The model under review builds one solid part; all positions refer to its coordinate system, in mm. Give positions to 0.01 mm unless a question says otherwise; leave off trailing zeros. Order: outer loops, then holes, each group sorted by start corner. A loop starts at its lowest first (then second) coordinate and runs counter-clockwise, first axis right, second up. Notation, with made-up numbers: (-18, 0.25) - (23, 0.25) arc R17 ccw to (23, 32.25) - close; hole circle Ø7 at (13.25, 10). An arc over 180 degrees is marked (long way). Use CSV: the item, a comma, the result in double quotes.
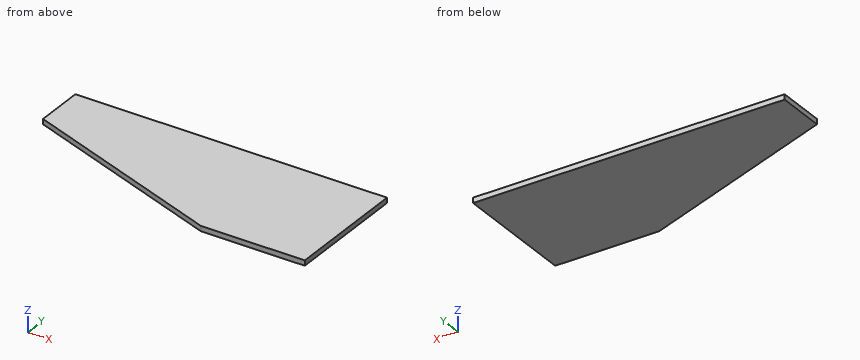
```python
from build123d import *

# Parameters (mm, degrees)
EXTRUDE_1_DEPTH = 5


with BuildPart() as part:
    # 草图1 → 凸台-拉伸1 (new body)
    with BuildSketch(Plane.XY):
        Polygon((0, 0), (300, 0), (300, -120), (200, -120), (0, -47.205953147), align=None)
    extrude(amount=EXTRUDE_1_DEPTH)


solid = part.part
```
Item 1: Take a section at C-C, the plane x = 64. Give the boundary of the cut face in (y, z), and give its area (4 significant figures).
Results list:
outline,"(-70.5, 0) - (0, 0) - (0, 5) - (-70.5, 5) - close"
area,"352.5 mm2"
Item 2: Take a section at B-B, the plane y = -58. Give the boundary of the cut face in (x, z).
Results list:
outline,"(29.66, 0) - (300, 0) - (300, 5) - (29.66, 5) - close"
Item 3: Wall thickness on L1, parallel to Y at x = 81, z = 3; L2, parallel to Y at x = 187, z = 4.3: over which ranges is each line inside the solid? List them lowest first.
Results list:
L1,"y = -76.69 to 0"
L2,"y = -115.27 to 0"
Item 4: Take a section at A-A, the plane z = 1.05. Give the boundary of the cut face in (x, y).
Results list:
outline,"(0, -47.21) - (200, -120) - (300, -120) - (300, 0) - (0, 0) - close"
Item 5: Clearance check with a flat-ended pin moving along its axis: pin 1 (1.5 mm diameter, centred on y = -25.5, z = 0.5, fed in from -X). State where the tip first meets the part, or that it passes through.
Results list:
pin 1,"stops at x = 0"
